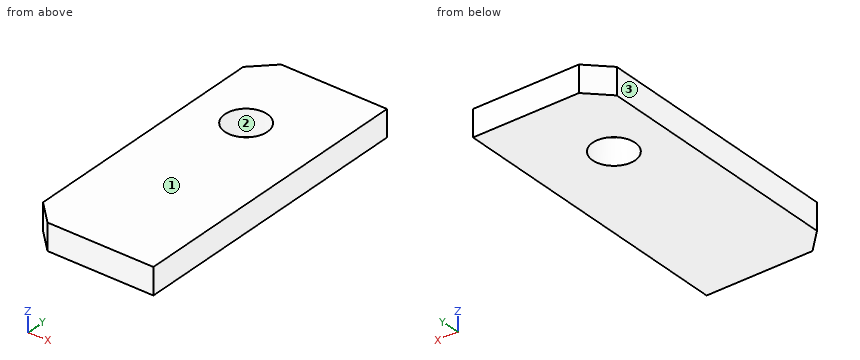
```python
from build123d import *

# Parameters (mm, degrees)
SKETCH_1_W               = 120
SKETCH_1_H               = 280
EXTRUDE_1_DEPTH          = 25
CUT_EXTRUDE_1_DEPTH      = 306.655034312
CUT_EXTRUDE_1_DEPTH_BACK = 306.655034312
SKETCH_2_R               = 20
CHAMFER_1_SIZE           = 20


with BuildPart() as part:
    # 草图1 → 凸台-拉伸1 (new body)
    with BuildSketch(Plane.XY):
        with Locations((-60, 140)):
            Rectangle(SKETCH_1_W, SKETCH_1_H)
    extrude(amount=EXTRUDE_1_DEPTH)

    # 草图2 → 切除-拉伸1 (cut, two sides: drawn at the far end of the back side and taken through both)
    with BuildSketch(Plane.XY.offset(25).offset(-CUT_EXTRUDE_1_DEPTH_BACK)):
        with Locations((-70, 200)):
            Circle(SKETCH_2_R)
    extrude(amount=CUT_EXTRUDE_1_DEPTH + CUT_EXTRUDE_1_DEPTH_BACK, mode=Mode.SUBTRACT)

    # 倒角1
    chamfer_1_edges = [part.edges().sort_by_distance(p)[0] for p in [
        (-120, 0, 12.5),
        (-120, 280, 12.5),
    ]]
    chamfer(chamfer_1_edges, length=CHAMFER_1_SIZE)


solid = part.part
```
CAD build for the part. Positions are in the model's coordinates, mm. Face numbers are marked on the shaded views. Round coordinates to 2 decimals unless told otherwise and drop trailing zeros. Order: outer loops, then holes, each group sorted by start corner. A loop starts at its lowest first (then second) coordinate and runs counter-clockwise, first axis right, second up. Notation, with made-up numbers: (29.5, -10.75) - (68.5, -10.75) arc R11 cw to (68.5, -6.75) - close; hole circle Ø3 at (1.5, -20). An arc over 180 degrees is marked (long way). Answer in a Markdown table with one row per item. Add a question column.
(1) Band-saw the part on B-B on x = -70. List the corners of the cut face in (y, z), and give its area (3 significant figures).
(2) Band-saw the part on A-A on y = 200. List the corners of the cut face in (x, z), and give its area (3 significant figures).
(3) Band-saw the part on C-C on z = 7.75. List the corners of the cut face in (x, y).
(4) Probe L1, parallel to X at y = 200, z = 8.25; L2, parallel to Y at x = -70, z = 15.5; L3, parallel to X at y = 192.5, z = 2. List the from-to ranges inside material, lowest first. Write a range as [from, to].
(5) Band-saw the part on D-D on x = -112. List the corners of the cut face in (y, z), and give its area (3 significant figures).
(6) Mould opens along X. For the marked faces 1, 2 and 3 say: +X half, -X half, draft (parallel to the pull), parting line (faces both ways), or undercut.
Data:
| question | item | result |
|---|---|---|
| 1 | outline | (0, 0) - (180, 0) - (180, 25) - (0, 25) - close; (220, 0) - (280, 0) - (280, 25) - (220, 25) - close |
| 1 | area | 6,000 mm^2 |
| 2 | outline | (-120, 0) - (-90, 0) - (-90, 25) - (-120, 25) - close; (-50, 0) - (0, 0) - (0, 25) - (-50, 25) - close |
| 2 | area | 2,000 mm^2 |
| 3 | outline | (-120, 20) - (-100, 0) - (0, 0) - (0, 280) - (-100, 280) - (-120, 260) - close; hole circle Ø40 at (-70, 200) |
| 4 | L1 | x = [-120, -90], [-50, 0] |
| 4 | L2 | y = [0, 180], [220, 280] |
| 4 | L3 | x = [-120, -88.54], [-51.46, 0] |
| 5 | outline | (12, 0) - (268, 0) - (268, 25) - (12, 25) - close |
| 5 | area | 6,400 mm^2 |
| 6 | face 1 | draft |
| 6 | face 2 | undercut |
| 6 | face 3 | -X half |
